Print and shaded views of the part. All mm, measured from the part's lowest x, y and z. Coordinates: 2 decimals unless noted, no trailing zeros. Order: outer loops, then holes, each group sorted by start corner. A loop starts at its lowest first (then second) coordinate and runs counter-clockwise, first axis right, second up. Notation, with made-up numbers: M 33.5,19.25 L 66.5,19.25 A18 ccw 66.5,39.25 Z; hole C 53.25,88 d8. An arc over 180 degrees is marked long. One line per item, written item: value.
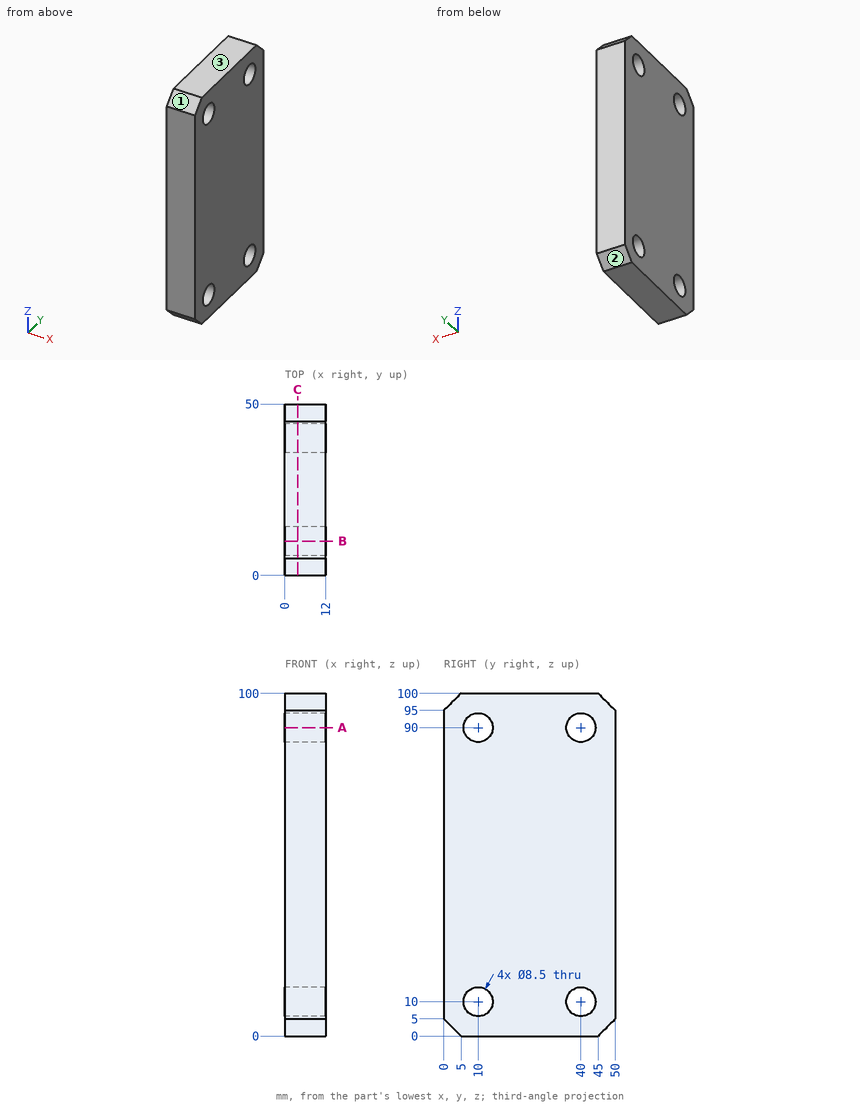
Q1. Drill centre lines: line 1 along Y through (x, z) = (9, 90); line 2 along Z through (x, y) = (11, 11); line 3 along Y through (x, z) = (11, 6.5). Where is each one in solid material? Low to high.
Recorded:
line 1: y = 0 to 5.75, 14.25 to 35.75, 44.25 to 50
line 2: z = 0 to 5.87, 14.13 to 85.87, 94.13 to 100
line 3: y = 0 to 7.59, 12.41 to 37.59, 42.41 to 50
Q2. Mould opens along Y. For the marked faces 1, 2 and 3 say: released by +Y, released by -Y, zero draft, split by the parting line, or undercut.
Recorded:
face 1: released by -Y
face 2: released by +Y
face 3: zero draft
Q3. Slice it at B-B (y = 10). List the corners of the cut face in (x, z).
Recorded:
outline: M 0,0 L 12,0 L 12,5.75 L 0,5.75 Z; M 0,14.25 L 12,14.25 L 12,85.75 L 0,85.75 Z; M 0,94.25 L 12,94.25 L 12,100 L 0,100 Z
Q4. Slice it at A-A (z = 90). List the corners of the cut face in (x, y).
Recorded:
outline: M 0,0 L 12,0 L 12,5.75 L 0,5.75 Z; M 0,14.25 L 12,14.25 L 12,35.75 L 0,35.75 Z; M 0,44.25 L 12,44.25 L 12,50 L 0,50 Z
Q5. Pin check, flat tip, straight feed: pin 1 Ø1 at (x, y) = (4, 41) entering from -Z. Stop position of the tip, or through.
Recorded:
pin 1: stops at z = 0
Q6. Slice it at C-C (x = 3.75). List the corners of the cut face in (y, z), plus the area to 3 significant figures.
Recorded:
outline: M 0,5 L 5,0 L 45,0 L 50,5 L 50,95 L 45,100 L 5,100 L 0,95 Z; hole C 10,10 d8.5; hole C 10,90 d8.5; hole C 40,10 d8.5; hole C 40,90 d8.5
area: 4,720 mm^2
